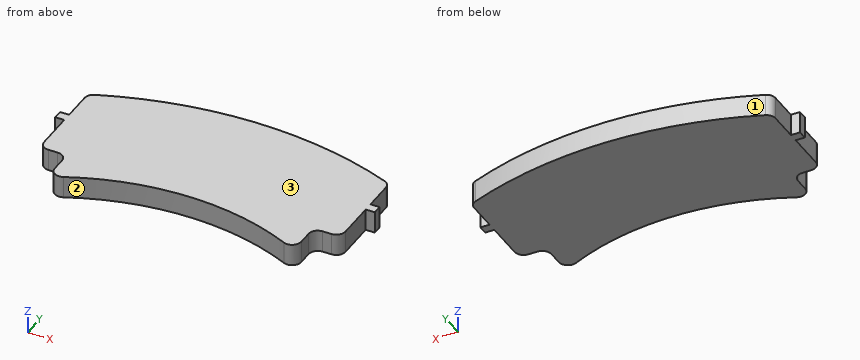
```python
from build123d import *

# Parameters (mm, degrees)
BOSS_EXTRUDE1_DEPTH = 6
SKETCH2_W           = 15
SKETCH2_H           = 30
CUT_EXTRUDE1_DEPTH  = 30
FILLET2_R           = 5
SKETCH3_W           = 5
SKETCH3_H           = 5
BOSS_EXTRUDE2_DEPTH = 12


with BuildPart() as part:
    # Sketch1 → Boss-Extrude1 (new, symmetric)
    with BuildSketch(Plane.XY):
        with BuildLine():
            Line((-82.5, 197.45822343), (-82.5, 116.802183199))
            ThreePointArc((-82.5, 116.802183199), (0, 143), (82.5, 116.802183199))
            Line((82.5, 116.802183199), (82.5, 197.45822343))
            ThreePointArc((82.5, 197.45822343), (0, 214), (-82.5, 197.45822343))
        make_face()
    extrude(amount=BOSS_EXTRUDE1_DEPTH, both=True)

    # Sketch2 → Cut-Extrude1 (cut)
    with BuildSketch(Plane.XY.offset(6)):
        with Locations((-75, 131.802183199)):
            Rectangle(SKETCH2_W, SKETCH2_H)
        with Locations((75, 131.802183199)):
            Rectangle(SKETCH2_W, SKETCH2_H)
    extrude(amount=-CUT_EXTRUDE1_DEPTH, mode=Mode.SUBTRACT)

    # Fillet2
    fillet2_edges = [part.edges().sort_by_distance(p)[0] for p in [
        (-82.5, 146.802183199, 0),
        (-67.5, 126.066450731, 0),
        (-67.5, 146.802183199, 0),
        (82.5, 146.802183199, 0),
        (67.5, 126.066450731, 0),
        (67.5, 146.802183199, 0),
        (-82.5, 197.45822343, 0),
        (82.5, 197.45822343, 0),
    ]]
    fillet(fillet2_edges, radius=FILLET2_R)

    # Sketch3 → Boss-Extrude2 (add)
    with BuildSketch(Plane.XY.offset(6)):
        with Locations((85, 175.45101432)):
            Rectangle(SKETCH3_W, SKETCH3_H)
        with Locations((-85, 175.45101432)):
            Rectangle(SKETCH3_W, SKETCH3_H)
    extrude(amount=-BOSS_EXTRUDE2_DEPTH)


solid = part.part
```
Work out the finished part from the listing and answer in its coordinate system (mm). Face numbers are marked on the shaded views. Give positions to 0.01 mm unless a question says otherwise; leave off trailing zeros. Order: outer loops, then holes, each group sorted by start corner. A loop starts at its lowest first (then second) coordinate and runs counter-clockwise, first axis right, second up.
1. Section C-C, the plane x = -15 is taken. Determine the outline of the cut face in (y, z).
Result sheet:
outline: (142.21, -6) - (213.47, -6) - (213.47, 6) - (142.21, 6) - close
2. The mould has two halves that part along X. Classify the marked faces 1, 2 and 3: released by +X, released by -X, zero draft, split by the parting line, or undercut.
Result sheet:
face 1: split by the parting line
face 2: undercut
face 3: zero draft
3. Section B-B, the plane y = 155.5 is taken. Determine the outline of the cut face in (x, z).
Result sheet:
outline: (-82.5, -6) - (82.5, -6) - (82.5, 6) - (-82.5, 6) - close
4. Each of these flat-tipped pins is pushed along its axis until it touches: P1, Ø2.5, axis at y = 139.5, z = 1, coming from the +X side; P2, Ø6, axis at y = 164.5, z = -0.5, coming from the -X side; P3, Ø1.5, axis at x = -85, z = 0.5, coming from the -Y side. Where does it stop, or does it pass through?
Result sheet:
P1: stops at x = 67.5
P2: stops at x = -82.5
P3: stops at y = 172.95
5. Straight lines are drawn through the part: L1, parallel to X at y = 160, z = 2.25; L2, parallel to Y at x = 41.5, z = -4.5; L3, parallel to X at y = 198.5, z = -3.25. For each, find the intervals that lie inside material, in ascending order.
Result sheet:
L1: x = -82.5 to 82.5
L2: y = 136.85 to 209.94
L3: x = -79.87 to 79.87
6. Section A-A, the plane z = 3 is taken. Determine the outline of the cut face in (x, y), and give its area (3 significant figures).
Result sheet:
outline: (-87.5, 172.95) - (-82.5, 172.95) - (-82.5, 151.8) arc R5 ccw to (-77.5, 146.8) - (-72.5, 146.8) arc R5 cw to (-67.5, 141.8) - (-67.5, 134.16) arc R5 ccw to (-60.39, 129.62) arc R143 cw to (60.39, 129.62) arc R5 ccw to (67.5, 134.16) - (67.5, 141.8) arc R5 cw to (72.5, 146.8) - (77.5, 146.8) arc R5 ccw to (82.5, 151.8) - (82.5, 172.95) - (87.5, 172.95) - (87.5, 177.95) - (82.5, 177.95) - (82.5, 194.1) arc R5 ccw to (79.35, 198.74) arc R214 ccw to (-79.35, 198.74) arc R5 ccw to (-82.5, 194.1) - (-82.5, 177.95) - (-87.5, 177.95) - close
area: 11,500 mm2
